Design review of the part built by this model. Coordinates are the model's own, in mm. Coordinates: 2 decimals unless noted, no trailing zeros. Loops run counter-clockwise (first coordinate to the right, second up) from the corner with the lowest first, then second, coordinate; pieces in that order, holes last. Notation, with made-up numbers: (61, 71.25) - (95, 71.25) arc R18 cw to (95, 82.25) - close; hole circle Ø6 at (45, 66). An arc over 180 degrees is marked (long way). Answer in a Markdown table with one row per item. Add a question column.
(1) We need section B-B, the plane z = 3.35. Write out the cut boundary in (x, y), plus the area to 3 significant figures.
(2) We need section C-C, the plane y = 0. Write out the cut boundary in (x, z), plus the area to 3 significant figures.
(3) We need section A-A, the plane x = -12. Write out the cut boundary in (y, z), plus the area to 3 significant figures.
(4) Clearance check with flat-ended pins moving along their axes: pin 1 (10.5 mm diameter, centred on x = -12, y = 0, fed in from +Z); pin 2 (6 mm diameter, centred on x = -41.5, y = 27.5, fed in from +Z). State where each tip first meets the part, or that it passes through.
(5) To check wall thickness, follow L1, parallel to X at y = 0, z = 0.5; L2, parallel to X at y = 0.5, z = 2.4; L3, parallel to Y at x = 46, z = 1.4. State the ranges of each line that lie inside material, in increasing order. Write a range as [from, to].
from build123d import *

# Parameters (mm, degrees)
SKETCH_1_W               = 120
SKETCH_1_H               = 68
EXTRUDE_1_DEPTH          = 4
HOLE_WIZARD_M6_1_D       = 5
FILLET_1_R               = 10
HOLE_WIZARD_3_AT_2_COUNT = 2
HOLE_WIZARD_3_AT_2_PITCH = 60


with BuildPart() as part:
    # 草图1 → 凸台-拉伸1 (new body)
    with BuildSketch(Plane.XY):
        Rectangle(SKETCH_1_W, SKETCH_1_H)
    extrude(amount=EXTRUDE_1_DEPTH)

    # M6 螺纹孔1 (through all)
    with Locations(Plane.XY.offset(4)):
        with Locations((28.49999693, -27.500007889), (-41.499997526, 27.499992111), (-41.499997526, -27.500007889), (28.49999693, 27.499992111)):
            Hole(HOLE_WIZARD_M6_1_D / 2)

    # 圆角1
    fillet_1_edges = [part.edges().sort_by_distance(p)[0] for p in [
        (60, -34, 2),
        (-60, -34, 2),
        (-60, 34, 2),
        (60, 34, 2),
    ]]
    fillet(fillet_1_edges, radius=FILLET_1_R)

    # 草图9 → 打孔尺寸(%根据)内六角花形半沉头螺钉的类型3 (revolve, cut)
    with BuildSketch(Plane(origin=(-12, 0, 4), x_dir=(0, -1, 0), z_dir=(1, 0, 0))):
        Polygon((0, 0), (0, 4), (3.3, 4), (3.3, 3.1), (6.4, 0), align=None)
    hole_wizard_3 = revolve(axis=Axis((-12, 0, 10.35), (0, 0, -1)), mode=Mode.SUBTRACT)

    # 打孔尺寸(%根据)内六角花形半沉头螺钉的类型3 at 2: 打孔尺寸(%根据)内六角花形半沉头螺钉的类型3 ×2
    with Locations(*[(i * HOLE_WIZARD_3_AT_2_PITCH, 0, 0) for i in range(1, HOLE_WIZARD_3_AT_2_COUNT)]):
        add(hole_wizard_3, mode=Mode.SUBTRACT)


solid = part.part
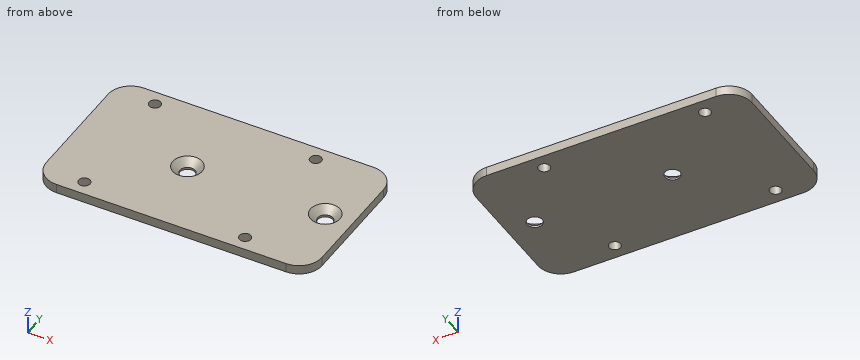
Responses:
| question | item | result |
|---|---|---|
| 1 | outline | (-60, -24) arc R10 ccw to (-50, -34) - (50, -34) arc R10 ccw to (60, -24) - (60, 24) arc R10 ccw to (50, 34) - (-50, 34) arc R10 ccw to (-60, 24) - close; hole circle Ø5 at (-41.5, -27.5); hole circle Ø5 at (-41.5, 27.5); hole circle Ø11.5 at (-12, 0); hole circle Ø5 at (28.5, -27.5); hole circle Ø5 at (28.5, 27.5); hole circle Ø11.5 at (48, 0) |
| 1 | area | 7,790 mm2 |
| 2 | outline | (-60, 0) - (-15.3, 0) - (-15.3, 0.9) - (-18.4, 4) - (-60, 4) - close; (-8.7, 0) - (44.7, 0) - (44.7, 0.9) - (41.6, 4) - (-5.6, 4) - (-8.7, 0.9) - close; (51.3, 0) - (60, 0) - (60, 4) - (54.4, 4) - (51.3, 0.9) - close |
| 2 | area | 408 mm2 |
| 3 | outline | (-34, 0) - (-3.3, 0) - (-3.3, 0.9) - (-6.4, 4) - (-34, 4) - close; (3.3, 0) - (34, 0) - (34, 4) - (6.4, 4) - (3.3, 0.9) - close |
| 3 | area | 236 mm2 |
| 4 | pin 1 | stops at z = 2.85 |
| 4 | pin 2 | stops at z = 4 |
| 5 | L1 | x = [-60, -15.3], [-8.7, 44.7], [51.3, 60] |
| 5 | L2 | x = [-60, -16.77], [-7.23, 43.23], [52.77, 60] |
| 5 | L3 | y = [-34, -3.23], [3.23, 34] |
